from build123d import *

# Parameters (mm, degrees)
ANCHOR_BLOCK_BODY_DEPTH             = 18.5
TOP_EDGE_CHAMFER_3X45_SIZE          = 3
STEP_GROOVE_DEPTH                   = 64.395583442
STEP_CUT_18_DEEP_DEPTH              = 27
COUNTERSUNK_THRU_HOLE_6_D           = 6
COUNTERSUNK_THRU_HOLE_6_CSINK_D     = 9
COUNTERSUNK_THRU_HOLE_6_CSINK_ANGLE = 90
DRILLED_HOLES_5X15_D                = 5
DRILLED_HOLES_5X15_DEPTH            = 12.5
DRILLED_HOLES_5X15_TIP              = 2.5


with BuildPart() as part:
    # Block Profile Sketch → Anchor Block Body (new, symmetric)
    with BuildSketch(Plane.XY):
        Polygon((0, 0), (0, 13), (7.498432223, 25), (15, 25), (15, 0), (43, 0), (43, -22), (45, -22), (45, -25), (0, -25), align=None)
    extrude(amount=ANCHOR_BLOCK_BODY_DEPTH, both=True)

    # Top Edge Chamfer 3x45
    top_edge_chamfer_3x45_edges = [part.edges().sort_by_distance(p)[0] for p in [
        (0, -25, 0),
    ]]
    chamfer(top_edge_chamfer_3x45_edges, length=TOP_EDGE_CHAMFER_3X45_SIZE)

    # Step Groove Sketch → Step Groove (cut, through all)
    with BuildSketch(Plane.XY.offset(18.5)):
        Polygon((12.878679656, -2.121320344), (12.171572875, -1.414213562), (15, 1.414213562), (16.414213562, 0), (13.585786438, -2.828427125), align=None)
    extrude(amount=-STEP_GROOVE_DEPTH, mode=Mode.SUBTRACT)

    # Step Cut Sketch → Step Cut 18 Deep (cut)
    with BuildSketch(Plane.ZY):
        with BuildLine():
            Line((-12, -25), (-12, -10.068287801))
            ThreePointArc((-12, -10.068287801), (0, -7), (12, -10.068287801))
            Line((12, -10.068287801), (12, -25))
            Line((12, -25), (-12, -25))
        make_face()
    extrude(amount=-STEP_CUT_18_DEEP_DEPTH, mode=Mode.SUBTRACT)

    # Countersunk Thru Hole Ø6 (through all)
    with Locations(Plane(origin=(43, 0, 0), x_dir=(0, 0, -1), z_dir=(1, 0, 0))):
        with Locations((0, -15)):
            CounterSinkHole(COUNTERSUNK_THRU_HOLE_6_D / 2, COUNTERSUNK_THRU_HOLE_6_CSINK_D / 2, counter_sink_angle=COUNTERSUNK_THRU_HOLE_6_CSINK_ANGLE)

    # Drilled Holes Ø5x15
    with Locations(Plane(origin=(43, 0, 0), x_dir=(0, 0, -1), z_dir=(1, 0, 0))):
        with Locations((12.5, -15), (-12.5, -15)):
            Hole(DRILLED_HOLES_5X15_D / 2, depth=DRILLED_HOLES_5X15_DEPTH)
            with Locations((0, 0, -(DRILLED_HOLES_5X15_DEPTH + DRILLED_HOLES_5X15_TIP / 2))):  # 90° drill point
                Cone(0, DRILLED_HOLES_5X15_D / 2, DRILLED_HOLES_5X15_TIP, mode=Mode.SUBTRACT)


solid = part.part
The listing builds one solid part. Answer for the finished solid, in the listing's coordinates (mm). A direction names the side the tool comes from. Give positions to 0.01 mm unless a question says otherwise; leave off trailing zeros. Loops run counter-clockwise (first coordinate to the right, second up) from the corner with the lowest first, then second, coordinate; pieces in that order, holes last.
Item 1: Each of these flat-tipped pins is pushed along its axis until it touches: pin 1 Ø1 at (x, z) = (44.5, 4) entering from +Y; pin 2 Ø6 at (y, z) = (5.5, 1.5) entering from -X; pin 3 Ø7 at (y, z) = (16.5, -7) entering from +X; pin 4 Ø2 at (y, z) = (16.5, 12) entering from -X. Where does it stop, or does it pass through?
Derived:
pin 1: stops at y = -22
pin 2: stops at x = 0
pin 3: stops at x = 15
pin 4: stops at x = 1.56
Item 2: Determine the mould class of faces 4 (the flat face through (15, 13, 0)), 5 (the flat face through (11, 25, 0)), 6 (the conical face through (28.71, -14.52, -11.98)) for opening direction Y: +Y half, -Y half, draft (parallel to the pull), parting line (faces both ways), or undercut.
Derived:
face 4: draft
face 5: +Y half
face 6: undercut
Item 3: A cutting plane is placed at C-C (x = 24). Give the vertices of the cut face in (y, z).
Derived:
outline: (-25, -18.5) - (0, -18.5) - (0, 18.5) - (-25, 18.5) - (-25, 12) - (-10.07, 12) arc R25 cw to (-10.07, -12) - (-25, -12) - close
Item 4: A cutting plane is placed at A-A (x = 32.5). Give the vertices of the cut face in (y, z), then the cut area to 3 significant figures.
Derived:
outline: (-25, -18.5) - (0, -18.5) - (0, 18.5) - (-25, 18.5) - close; hole circle Ø6 at (-15, 0); hole circle Ø5 at (-15, -12.5); hole circle Ø5 at (-15, 12.5)
area: 857 mm2
Item 5: Find the intervals of material crossed by line 1 along Z through (x, y) = (37.25, -15); line 2 along Y through (x, z) = (39, 12.5); line 3 along Z through (x, y) = (8, -22), in increasing order.
Derived:
line 1: z = -18.5 to -15, -10 to -3, 3 to 10, 15 to 18.5
line 2: y = -25 to -17.5, -12.5 to 0
line 3: z = -18.5 to -12, 12 to 18.5
Item 6: A cutting plane is placed at D-D (z = 9). Give the vertices of the cut face in (x, y), then the cut area to 3 significant figures.
Derived:
outline: (0, -8.68) - (27, -8.68) - (27, -25) - (45, -25) - (45, -22) - (43, -22) - (43, 0) - (16.41, 0) - (13.59, -2.83) - (12.17, -1.41) - (15, 1.41) - (15, 25) - (7.5, 25) - (0, 13) - close
area: 963 mm2
Item 7: A cutting plane is placed at B-B (z = 0). Give the vertices of the cut face in (x, y), then the cut area to 3 significant figures.
Derived:
outline: (0, -7) - (27, -7) - (27, -12) - (41.5, -12) - (43, -10.5) - (43, 0) - (16.41, 0) - (13.59, -2.83) - (12.17, -1.41) - (15, 1.41) - (15, 25) - (7.5, 25) - (0, 13) - close; (27, -25) - (45, -25) - (45, -22) - (43, -22) - (43, -19.5) - (41.5, -18) - (27, -18) - close
area: 820 mm2
Item 8: A tool of negligible diameter and unlimited length cuts with its end or side. For faces 1 (the flat face through (43, -8, 0)), 2 (the cylindrical face through (37, -15, 10)), 3 (the cylindrical face through (13, -7, 0)), from which of +Z, -Z, +X, -X, +Y, -Y can it reach the whole face along a straight path? Write none if from no direction.
Derived:
face 1: +Z, -Z, +X, +Y
face 2: +X
face 3: -X, -Y
